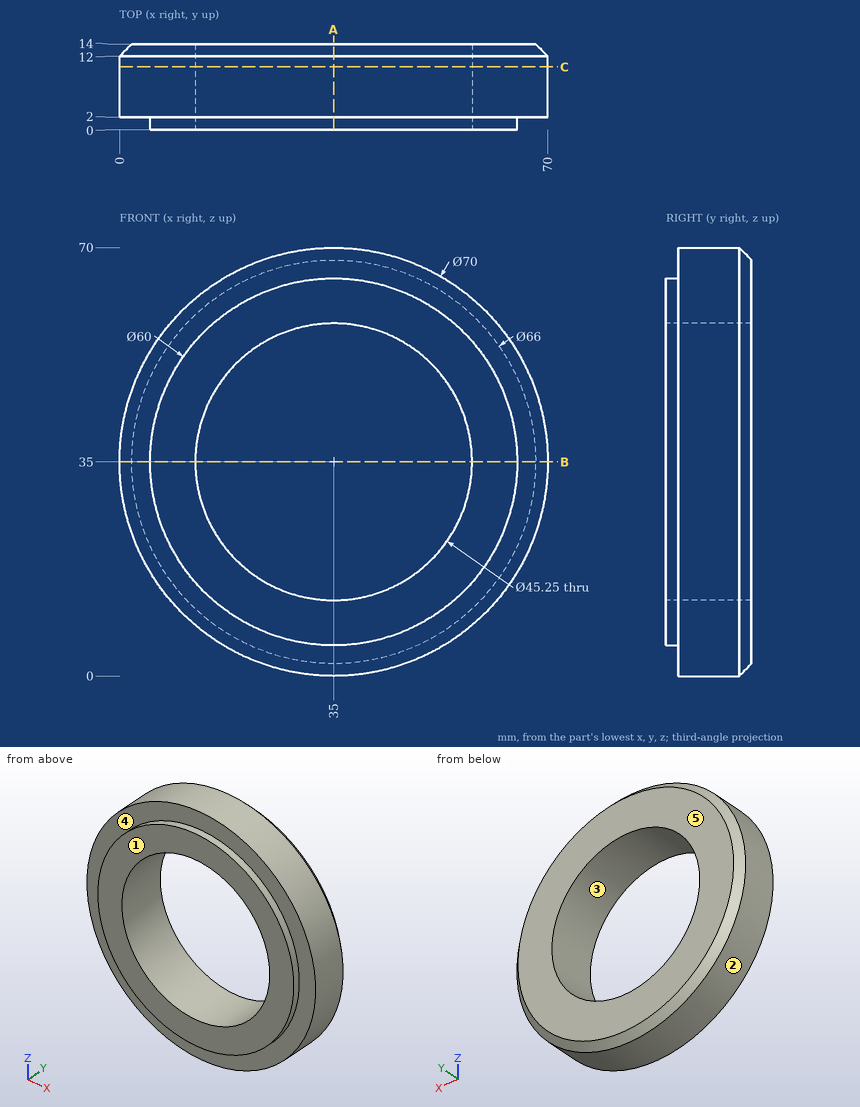
Check sheet for the drawn part. Datum: minimum x, y, z corner. Units: mm. A direction names the side the tool comes from. Round coordinates to 2 decimals unless told otherwise and drop trailing zeros. Order: outer loops, then holes, each group sorted by start corner. A loop starts at its lowest first (then second) coordinate and runs counter-clockwise, first axis right, second up.
(1) Scan lines: probe 1 along Z at (x, y) = (35, 9) (3 decimals); probe 2 along Z at (x, y) = (15, 11.5); probe 3 along X at (y, z) = (8, 21). Record each from-to range of solid material in increasing order.
(2) Cross-section at C-C, the plane y = 10.25. Enter the section's corners in (x, z) (3 decimals).
(3) Cross-section at A-A, the plane x = 35. Enter the section's corners in (y, z) (3 decimals), and give its area (4 significant figures).
(4) Access from +Z, -Z, +X, -X, +Y, -Y to the whole of each face (thin tool, end or side, straight path). Record for the marked faces 4 and 5.
(5) Draft check along X on the marked faces 1, 2 and 3. Enter one of: pulls with the +X half, pulls with the -X half, needs draft (parallel to the pull), parting line crosses it, or undercut.
(6) Cross-section at B-B, the plane z = 35. Enter the section's corners in (x, y) (3 decimals), and give its area (4 significant figures).
(7) Go/stop test with flat-tipped pins: P1, Ø5, axis at x = 17.5, y = 7.5, coming from the -Z side; P2, Ø6, axis at x = 47.5, y = 1.5, coming from the -Z side; P3, Ø1.5, axis at x = 18.5, y = 11, coming from the -Z side. Record where each tip stops, or that it passes through.
Check sheet entries:
1. probe 1: z = 0 to 12.375, 57.625 to 70
1. probe 2: z = 6.28 to 24.42, 45.58 to 63.72
1. probe 3: x = 2.92 to 17.23, 52.77 to 67.08
2. outline: circle Ø70 at (35, 35); hole circle Ø45.25 at (35, 35)
3. outline: (0, 5) - (2, 5) - (2, 0) - (12, 0) - (14, 2) - (14, 12.375) - (0, 12.375) - close; (0, 57.625) - (14, 57.625) - (14, 68) - (12, 70) - (2, 70) - (2, 65) - (0, 65) - close
3. area: 322.5 mm2
4. face 4: -Y
4. face 5: +Z, -Z, +X, -X, +Y
5. face 1: needs draft
5. face 2: parting line crosses it
5. face 3: undercut
6. outline: (0, 2) - (5, 2) - (5, 0) - (12.375, 0) - (12.375, 14) - (2, 14) - (0, 12) - close; (57.625, 0) - (65, 0) - (65, 2) - (70, 2) - (70, 12) - (68, 14) - (57.625, 14) - close
6. area: 322.5 mm2
7. P1: stops at z = 3.38
7. P2: stops at z = 1.33
7. P3: stops at z = 3.74
